from build123d import *

# Parameters (mm, degrees)
END_CHAMFERS_3X45_SIZE = 3


with BuildPart() as part:
    # Pin Profile Sketch → Pin Body Revolve (revolve)
    with BuildSketch(Plane.XY, mode=Mode.PRIVATE) as pin_body_revolve_sk:
        Polygon((0, 131.5), (9.5, 131.5), (9.5, 81.5), (13, 81.5), (13, -81.5), (9.5, -81.5), (9.5, -131.5), (0, -131.5), align=None)
    revolve(pin_body_revolve_sk.sketch.rotate(Axis((0, 65.559405941, 0), (0, -1, 0)), 90), axis=Axis((0, 65.559405941, 0), (0, -1, 0)))

    # End Chamfers 3x45°
    end_chamfers_3x45_edges = [part.edges().sort_by_distance(p)[0] for p in [
        (0, -131.5, -9.5),
        (0, 131.5, -9.5),
    ]]
    chamfer(end_chamfers_3x45_edges, length=END_CHAMFERS_3X45_SIZE)


solid = part.part
Can you work these out from the model? Positions are in its coordinate system, mm. A direction names the side the tool comes from. Coordinates: 2 decimals unless noted, no trailing zeros. Write each loop counter-clockwise with the first axis right and the second up, starting at its lowest first coordinate (ties: lowest second). Pieces come first, ordered by that corner, then holes. Notation, with made-up numbers: (-22, 81.5) - (-15, 81.5) arc R24 ccw to (-15, 111.5) - close; hole circle Ø8 at (-3.5, -38). An arc over 180 degrees is marked (long way). Return JSON: item names as keys, results as strings. Group by question number.
Item 1: If we section it at B-B (x = 0): Write out the boundary of the cut face in (y, z).
Item 2: Which directions (+Z, -Z, +X, -X, +Y, -Y) give clear straight access to the entire face, cutting with the end or side of a thin tool? Please do faces 1 (the face through (9.274, -105.329, -2.059)), 2 (the face through (9.274, 104.671, -2.059)), 3 (the face through (7.91, -1.141, -10.316)).
Item 3: If we section it at D-D (y = 89): Write out the boundary of the cut face in (x, z).
Item 4: If we section it at C-C (y = -37.5): Write out the boundary of the cut face in (x, z), then the cut area to 3 significant figures.
Item 5: I'm going to push flat-ended pins straight in: pin 1 Ø6 at (x, y) = (-4.5, -102) entering from +Z; pin 2 Ø2 at (x, z) = (9, 2) entering from +Y; pin 3 Ø2 at (y, z) = (72.5, -3.5) entering from +X; pin 4 Ø12 at (x, z) = (3.5, 6) entering from +Y. Where does each tip first touch, or does it pass through?
Item 6: If we section it at A-A (z = 0): Write out the boundary of the cut face in (x, y).
Item 7: Please list where these lines run through material, in increasing order: probe 1 along Y at (x, z) = (7, 10.25); probe 2 along X at (y, z) = (-84.5, -0.25); probe 3 along X at (y, z) = (-54, 11.75).
Return value:
{
 "1": {"outline": "(-131.5, -6.5) - (-128.5, -9.5) - (-81.5, -9.5) - (-81.5, -13) - (81.5, -13) - (81.5, -9.5) - (128.5, -9.5) - (131.5, -6.5) - (131.5, 6.5) - (128.5, 9.5) - (81.5, 9.5) - (81.5, 13) - (-81.5, 13) - (-81.5, 9.5) - (-128.5, 9.5) - (-131.5, 6.5) - close"},
 "2": {"face 1": "-Y", "face 2": "+Y", "face 3": "+Y, -Y"},
 "3": {"outline": "circle Ø19 at (0, 0)"},
 "4": {"outline": "circle Ø26 at (0, 0)", "area": "531 mm^2"},
 "5": {"pin 1": "stops at z = 9.38", "pin 2": "stops at y = 129.78", "pin 3": "stops at x = 12.76", "pin 4": "stops at y = 131.5"},
 "6": {"outline": "(-13, -81.5) - (-9.5, -81.5) - (-9.5, -128.5) - (-6.5, -131.5) - (6.5, -131.5) - (9.5, -128.5) - (9.5, -81.5) - (13, -81.5) - (13, 81.5) - (9.5, 81.5) - (9.5, 128.5) - (6.5, 131.5) - (-6.5, 131.5) - (-9.5, 128.5) - (-9.5, 81.5) - (-13, 81.5) - close"},
 "7": {"probe 1": "y = -81.5 to 81.5", "probe 2": "x = -9.5 to 9.5", "probe 3": "x = -5.56 to 5.56"}
}
